Could you check a few things on this model? Use its own coordinates, in mm. A direction names the side the tool comes from. Round coordinates to 2 decimals unless told otherwise and drop trailing zeros. Write each loop counter-clockwise with the first axis right and the second up, starting at its lowest first coordinate (ties: lowest second). Pieces come first, ordered by that corner, then holes. Notation, with made-up numbers: (5, 43) - (12, 43) arc R13 ccw to (12, 64) - close; hole circle Ø11 at (49.5, 30). An arc over 180 degrees is marked (long way). Put each result on its own line as item: value.
from build123d import *

# Parameters (mm, degrees)
SKETCH_1_W                   = 25
SKETCH_1_H                   = 25
EXTRUDE_1_DEPTH              = 10
CHAMFER_1_SIZE               = 2
HOLE_WIZARD_M6_1_D           = 5
HOLE_WIZARD_M4_1_D           = 4.5
HOLE_WIZARD_M4_1_CBORE_D     = 8
HOLE_WIZARD_M4_1_CBORE_DEPTH = 19.6


with BuildPart() as part:
    # 草图1 → 凸台-拉伸1 (new body)
    with BuildSketch(Plane(origin=(0, 0, 0), x_dir=(1, 0, 0), z_dir=(0, 1, 0))):
        Rectangle(SKETCH_1_W, SKETCH_1_H)
    extrude(amount=EXTRUDE_1_DEPTH)

    # 倒角1
    chamfer_1_edges = [part.edges().sort_by_distance(p)[0] for p in [
        (-12.5, 5, -12.5),
        (12.5, 5, -12.5),
    ]]
    chamfer(chamfer_1_edges, length=CHAMFER_1_SIZE)

    # M6 螺纹孔1 (through all)
    with Locations(Plane(origin=(0, 0, 0), x_dir=(-1, 0, 0), z_dir=(0, -1, 0))):
        with Locations((0, 0)):
            Hole(HOLE_WIZARD_M6_1_D / 2)

    # M4 六角圆柱头螺钉的柱形沉头孔1 (through all)
    with Locations(Plane(origin=(0, 0, -12.5), x_dir=(-1, 0, 0), z_dir=(0, 0, -1))):
        with Locations((-7.5, 5), (7.5, 5)):
            CounterBoreHole(HOLE_WIZARD_M4_1_D / 2, HOLE_WIZARD_M4_1_CBORE_D / 2, HOLE_WIZARD_M4_1_CBORE_DEPTH)


solid = part.part
(1) For faces 4 (the face through (6, 3, 7.1)), 5 (the face through (-9.16, 6.52, 9.84)), which set-ups out of +Z, -Z, +X, -X, +Y, -Y let a thin tool reach every point of the face, with its end or its side?
Values found:
face 4: -Z
face 5: +Z, -Z
(2) Imagine slicing it at D-D, the plane z = -3. List the corners of the cut face in (x, y) for me, then the cut area to 3 significant figures.
Values found:
outline: (-12.5, 0) - (12.5, 0) - (12.5, 10) - (-12.5, 10) - close; hole circle Ø8 at (-7.5, 5); hole circle Ø8 at (7.5, 5)
area: 149 mm^2
(3) Imagine slicing it at C-C, the plane y = 4. List the corners of the cut face in (x, z) for me.
Values found:
outline: (-12.5, -10.5) - (-11.37, -11.63) - (-11.37, 7.1) - (-9.52, 7.1) - (-9.52, 12.5) - (-12.5, 12.5) - close; (-5.48, 7.1) - (-3.63, 7.1) - (-3.63, -12.5) - (3.63, -12.5) - (3.63, 7.1) - (5.48, 7.1) - (5.48, 12.5) - (-5.48, 12.5) - close; (9.52, 7.1) - (11.37, 7.1) - (11.37, -11.63) - (12.5, -10.5) - (12.5, 12.5) - (9.52, 12.5) - close; hole circle Ø5 at (0, 0)
(4) Please list where these lines run through material, in increasing order: probe 1 along Z at (x, y) = (0, 5); probe 2 along X at (y, z) = (5.5, -6.5); probe 3 along X at (y, z) = (4, -3.5). Write a range as from..to.
Values found:
probe 1: z = -12.5..-2.5, 2.5..12.5
probe 2: x = -12.5..-11.47, -3.53..3.53, 11.47..12.5
probe 3: x = -12.5..-11.37, -3.63..3.63, 11.37..12.5
(5) Imagine slicing it at B-B, the plane x = 0. List the corners of the cut face in (y, z) for me.
Values found:
outline: (0, -12.5) - (10, -12.5) - (10, -2.5) - (0, -2.5) - close; (0, 2.5) - (10, 2.5) - (10, 12.5) - (0, 12.5) - close
(6) If we mould it in two halves opening along X, with no side actions, what happens to faces 1 (the face through (5.84, 6.52, 9.84)), 2 (the face through (0, 0, -3)), 3 (the face through (-12, 5, -11))? For each: pulls with the +X half, pulls with the -X half, needs draft (parallel to the pull), parting line crosses it, or undercut.
Values found:
face 1: undercut
face 2: needs draft
face 3: pulls with the -X half
(7) Imagine slicing it at A-A, the plane z = 0. List the corners of the cut face in (x, y) for me.
Values found:
outline: (-12.5, 0) - (-2.5, 0) - (-2.5, 10) - (-12.5, 10) - close; (2.5, 0) - (12.5, 0) - (12.5, 10) - (2.5, 10) - close; hole circle Ø8 at (-7.5, 5); hole circle Ø8 at (7.5, 5)
